Verification items for the finished model (mm, model axes). Face numbers are marked on the shaded views. A direction names the side the tool comes from. Coordinates: 2 decimals unless noted, no trailing zeros. Order: outer loops, then holes, each group sorted by start corner. A loop starts at its lowest first (then second) coordinate and runs counter-clockwise, first axis right, second up. Notation, with made-up numbers: M 56,21.25 L 90,21.25 A21 cw 90,42.25 Z; hole C 80.5,81.5 d9. An arc over 180 degrees is marked long. Answer as a JSON object with one key per item and string values. Group by question number.
(1) Cross-section at B-B (x = 6.5). Enter the section's corners in (y, z), plus the area to 3 significant figures.
(2) Material ranges on line 1 (Y direction, x = 15.75, z = 0); line 2 (Y direction, x = 9, z = 0); line 3 (X direction, y = -39, z = -57), recorded low to high.
(3) Access from +Z, -Z, +X, -X, +Y, -Y to the whole of each face (thin tool, end or side, straight path). Record for the marked faces 4 and 5.
(4) Cross-section at A-A (z = 0). Enter the section's corners in (x, y), plus the area to 3 significant figures.
(5) Gauge pin test, flat ends, axial feed: pin 1 Ø1.5 at (x, z) = (8.5, 53) entering from +Y; pin 2 Ø10 at (x, z) = (3.5, -11.5) entering from +Y; pin 3 Ø7.5 at (y, z) = (-70, 0) entering from -X; pin 4 Ø4 at (x, y) = (6, 7.5) entering from -Z. Record the tip position at first contact, or that the pin passes through.
(6) Mould release check, pull along Y, two halves, no side actions. Record for the marked faces 1, 2 and 3: released by +Y, released by -Y, zero draft, split by the parting line, or undercut.
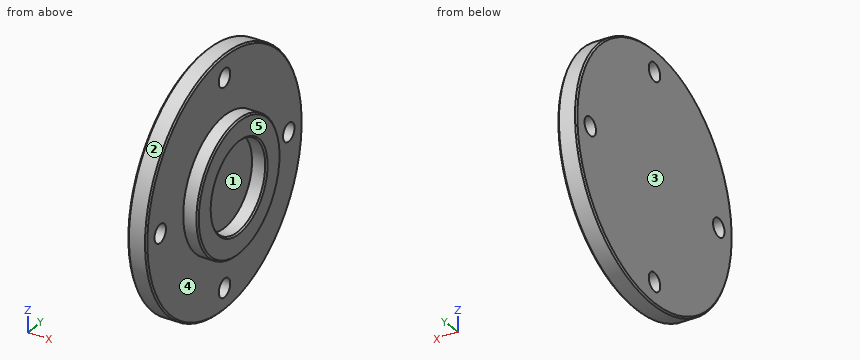
from build123d import *

# Parameters (mm, degrees)
SKETCH_2_R               = 6.25
CUT_EXTRUDE_1_DEPTH      = 123.388724971
PATTERN_CIRCULAR_1_COUNT = 4
CHAMFER_1_SIZE           = 1


with BuildPart() as part:
    # 草图1 → 旋转1 (revolve)
    with BuildSketch(Plane.XY, mode=Mode.PRIVATE) as revolve_1_sk:
        Polygon((0, 0), (0, 85), (13, 85), (13, 45), (23, 45), (23, 30), (13, 30), (13, 0), align=None)
    revolve(revolve_1_sk.sketch.rotate(Axis((0, 0, 0), (1, 0, 0)), 90), axis=Axis((0, 0, 0), (1, 0, 0)))

    # 草图2 → 切除-拉伸1 (cut, through all)
    with BuildSketch(Plane.ZY):
        with Locations((0, 70)):
            Circle(SKETCH_2_R)
    cut_extrude_1 = extrude(amount=-CUT_EXTRUDE_1_DEPTH, mode=Mode.SUBTRACT)

    # 阵列(圆周)1: 切除-拉伸1 ×4 about axis
    pattern_circular_1_axis = Axis((0, 0, 0), (1, 0, 0))
    for i in range(1, PATTERN_CIRCULAR_1_COUNT):
        add(cut_extrude_1.rotate(pattern_circular_1_axis, i * 360 / PATTERN_CIRCULAR_1_COUNT), mode=Mode.SUBTRACT)

    # 倒角1
    chamfer_1_edges = [part.edges().sort_by_distance(p)[0] for p in [
        (23, 0, -30),
        (23, 0, -45),
        (13, 0, -85),
        (0, 0, -85),
    ]]
    chamfer(chamfer_1_edges, length=CHAMFER_1_SIZE)


solid = part.part
Taken from the geometry:
{
 "1": {"outline": "C 0,0 d170; hole C -70,0 d12.5; hole C 0,-70 d12.5; hole C 0,70 d12.5; hole C 70,0 d12.5", "area": "22,200 mm²"},
 "2": {"line 1": "y = -45 to -30, 30 to 45", "line 2": "y = -85 to -76.25, -63.75 to 63.75, 76.25 to 85", "line 3": "x = 0 to 13"},
 "3": {"face 4": "+X", "face 5": "+Z, -Z, +X, +Y, -Y"},
 "4": {"outline": "M 0,-84 L 1,-85 L 12,-85 L 13,-84 L 13,-76.25 L 0,-76.25 Z; M 0,-63.75 L 13,-63.75 L 13,-45 L 22,-45 L 23,-44 L 23,-31 L 22,-30 L 13,-30 L 13,30 L 22,30 L 23,31 L 23,44 L 22,45 L 13,45 L 13,63.75 L 0,63.75 Z; M 0,76.25 L 13,76.25 L 13,84 L 12,85 L 1,85 L 0,84 Z", "area": "2,180 mm²"},
 "5": {"pin 1": "stops at y = 67.04", "pin 2": "stops at y = 84.75", "pin 3": "passes through", "pin 4": "stops at z = -84.82"},
 "6": {"face 1": "undercut", "face 2": "split by the parting line", "face 3": "zero draft"}
}
